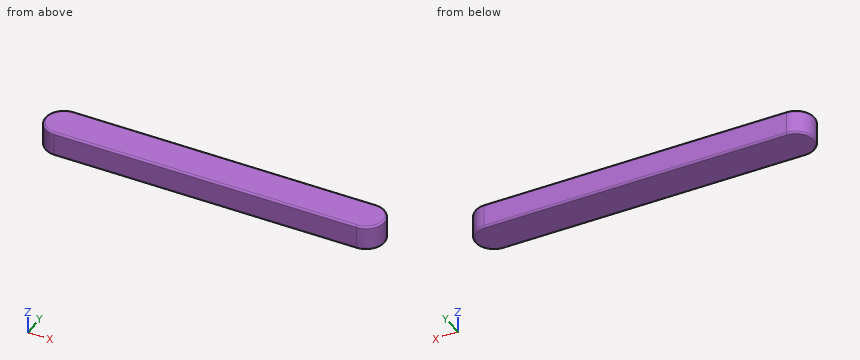
```python
from build123d import *

# Parameters (mm, degrees)
EXTRUDE_523_DEPTH = 8
FILLET_1_R        = 0.6


with BuildPart() as part:
    # 草图1 → Extrude 523 (new body)
    with BuildSketch(Plane.XY):
        with BuildLine():
            Line((-49, 6), (49, 6))
            ThreePointArc((49, 6), (55, 0), (49, -6))
            Line((49, -6), (-49, -6))
            ThreePointArc((-49, -6), (-55, 0), (-49, 6))
        make_face()
    extrude(amount=EXTRUDE_523_DEPTH)

    # 圆角1
    fillet_1_edges = [part.edges().sort_by_distance(p)[0] for p in [
        (55, 0, 8),
        (0, 6, 8),
        (-55, 0, 8),
        (0, 6, 0),
        (55, 0, 0),
        (0, -6, 0),
        (-55, 0, 0),
        (0, -6, 8),
    ]]
    fillet(fillet_1_edges, radius=FILLET_1_R)


solid = part.part
```
Here's how the part is built. I have some questions about the finished solid (model axes, mm). Round coordinates to 2 decimals unless told otherwise and drop trailing zeros. Write each loop counter-clockwise with the first axis right and the second up, starting at its lowest first coordinate (ties: lowest second). Pieces come first, ordered by that corner, then holes.
Q1. Please list where these lines run through material, in increasing order: probe 1 along X at (y, z) = (-0.5, 3.25); probe 2 along X at (y, z) = (-2.75, 3.25); probe 3 along Y at (x, z) = (50.5, 4.5).
Q2. Will this pin go through, and if not, where does the flat tip stop? P1, Ø2, axis at y = -5, z = 1.5, coming from the -X side.
Q3. If we section it at A-A on z = 3.5: Write out the boundary of the cut face in (x, y), plus the area to 3 significant figures.
Answer below:
1. probe 1: x = -54.98 to 54.98
1. probe 2: x = -54.33 to 54.33
1. probe 3: y = -5.81 to 5.81
2. P1: stops at x = -53.47
3. outline: (-49, -6) - (49, -6) arc R6 ccw to (49, 6) - (-49, 6) arc R6 ccw to start
3. area: 1,290 mm2
